For this review, take the finished solid that the model builds, in its own axes (mm). Coordinates: 2 decimals unless noted, no trailing zeros. Loops run counter-clockwise (first coordinate to the right, second up) from the corner with the lowest first, then second, coordinate; pieces in that order, holes last. Notation, with made-up numbers: (29, 62) -> (62, 62) arc R28 ccw to (62, 84) -> close; hole circle Ø9 at (8.25, -1.75). An arc over 180 degrees is marked (long way). One line per item, written item: value.
from build123d import *

# Parameters (mm, degrees)
BOSS_EXTRUDE1_DEPTH = 40
SKETCH2_R           = 47.5
CUT_EXTRUDE1_DEPTH  = 284.240180765
M16_TAPPED_HOLE1_D  = 14


with BuildPart() as part:
    # Sketch1 → Boss-Extrude1 (new body)
    with BuildSketch(Plane.XY):
        with BuildLine():
            Line((-215, -180), (215, -180))
            Line((215, -180), (215, -65))
            Line((215, -65), (90.722959932, 78.545175161))
            ThreePointArc((90.722959932, 78.545175161), (0, 120), (-90.722959932, 78.545175161))
            Line((-90.722959932, 78.545175161), (-215, -65))
            Line((-215, -65), (-215, -180))
        make_face()
    extrude(amount=BOSS_EXTRUDE1_DEPTH)

    # Sketch2 → Cut-Extrude1 (cut, through all)
    with BuildSketch(Plane.XY.offset(40)):
        Circle(SKETCH2_R)
    extrude(amount=-CUT_EXTRUDE1_DEPTH, mode=Mode.SUBTRACT)

    # M16 Tapped Hole1 (through all)
    with Locations(Plane.XY.offset(40)):
        with Locations((-110, -120), (110, -120)):
            Hole(M16_TAPPED_HOLE1_D / 2)


solid = part.part
1. Take a section at A-A, the plane x = 0. Give the boundary of the cut face in (y, z), and give its area (3 significant figures).
Return value:
outline: (-180, 0) -> (-47.5, 0) -> (-47.5, 40) -> (-180, 40) -> close; (47.5, 0) -> (120, 0) -> (120, 40) -> (47.5, 40) -> close
area: 8,200 mm2
2. Insertion check: pin 1 Ø1.5 at (x, y) = (31.5, -142) entering from -Z; pin 2 Ø6 at (y, z) = (-42.5, 8.5) entering from +X; pin 3 Ø1 at (x, z) = (-11, 27.5) entering from +Y; pin 4 Ø1 at (y, z) = (13, 32) entering from +X. Each pin has a flat end and moves straight along its axis. Give the tip position at first contact, or say it passes through.
Return value:
pin 1: stops at z = 0
pin 2: stops at x = 198.12
pin 3: stops at y = 119.54
pin 4: stops at x = 147.9
3. Take a section at D-D, the plane x = 62. Give the boundary of the cut face in (y, z), and give its area (3 significant figures).
Return value:
outline: (-180, 0) -> (102.74, 0) -> (102.74, 40) -> (-180, 40) -> close
area: 11,300 mm2
4. Take a section at C-C, the plane z = 27.5. Give the boundary of the cut face in (x, y), and give its area (3 significant figures).
Return value:
outline: (-215, -180) -> (215, -180) -> (215, -65) -> (90.72, 78.55) arc R120 ccw to (-90.72, 78.55) -> (-215, -65) -> close; hole circle Ø14 at (-110, -120); hole circle Ø95 at (0, 0); hole circle Ø14 at (110, -120)
area: 91,200 mm2
5. To check wall thickness, follow probe 1 along X at (y, z) = (41, 37); probe 2 along Y at (x, z) = (-37, 18.5); probe 3 along Y at (x, z) = (31, 9.5). State the ranges of each line that lie inside material, in increasing order. Write a range as from..to.
Return value:
probe 1: x = -123.23..-23.98, 23.98..123.23
probe 2: y = -180..-29.79, 29.79..114.15
probe 3: y = -180..-35.99, 35.99..115.93
6. Take a section at B-B, the plane y = 12. Give the boundary of the cut face in (x, z).
Return value:
outline: (-148.34, 0) -> (-45.96, 0) -> (-45.96, 40) -> (-148.34, 40) -> close; (45.96, 0) -> (148.34, 0) -> (148.34, 40) -> (45.96, 40) -> close
